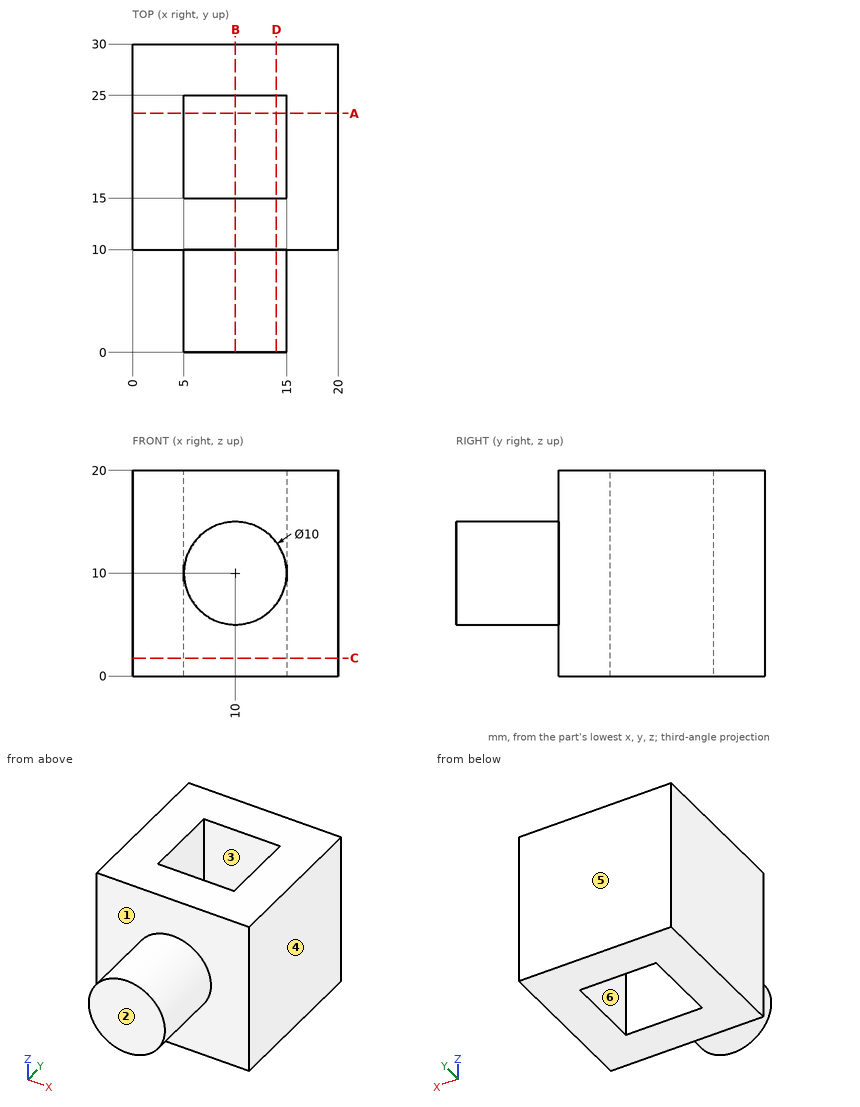
The drawing under review shows one solid part. Ordinate dimensions are in mm from its lowest x, y, z. A direction names the side the tool comes from. Round coordinates to 2 decimals unless told otherwise and drop trailing zeros. Write each loop counter-clockwise with the first axis right and the second up, starting at its lowest first coordinate (ties: lowest second). Pieces come first, ordered by that corner, then holes. Notation, with made-up numbers: (79, 58) - (119, 58) arc R23 cw to (119, 74) - close; hole circle Ø11 at (14.25, 10.25). An arc over 180 degrees is marked (long way). Use one line per item in the form item = value.
Q1. For line 1 (X direction, y = 20.75, z = 11); line 2 (Y direction, x = 9, z = 14); line 3 (Y direction, x = 7, z = 5.5), list the stretches that pass through material, from the lowest coordinate up. Write a range as [from, to].
Answer key:
line_1 = [0, 5], [15, 20]
line_2 = [0, 15], [25, 30]
line_3 = [10, 15], [25, 30]
Q2. Consider section C-C (z = 1.75). State the section outline as (x, y) points, and give its area (3 significant figures).
Answer key:
outline = (0, 10) - (20, 10) - (20, 30) - (0, 30) - close; hole (5, 15) - (15, 15) - (15, 25) - (5, 25) - close
area = 300 mm2
Q3. Consider section D-D (x = 14). State the section outline as (y, z) points.
Answer key:
outline = (0, 7) - (10, 7) - (10, 0) - (15, 0) - (15, 20) - (10, 20) - (10, 13) - (0, 13) - close; (25, 0) - (30, 0) - (30, 20) - (25, 20) - close
Q4. Insertion check: pin 1 Ø3 at (x, y) = (9, 17) entering from +Z. The pin has a flat end and moves straight along its axis. Give the tip position at first contact, or say it passes through.
Answer key:
pin_1 = through
Q5. Draft analysis for pull direction Y (two halves, no side actions). For the marked faces 4, 5 and 6, state which applies: +Y half, -Y half, draft (parallel to the pull), parting line (faces both ways), or undercut.
Answer key:
face_4 = draft
face_5 = +Y half
face_6 = undercut
Q6. Consider section A-A (y = 23.25). State the section outline as (x, z) points.
Answer key:
outline = (0, 0) - (5, 0) - (5, 20) - (0, 20) - close; (15, 0) - (20, 0) - (20, 20) - (15, 20) - close
Q7. Consider section B-B (x = 10). State the section outline as (y, z) points, and give its area (3 significant figures).
Answer key:
outline = (0, 5) - (10, 5) - (10, 0) - (15, 0) - (15, 20) - (10, 20) - (10, 15) - (0, 15) - close; (25, 0) - (30, 0) - (30, 20) - (25, 20) - close
area = 300 mm2
Q8. Tool access review of the marked faces 1, 2 and 3: name each direction out of +Z, -Z, +X, -X, +Y, -Y from which nothing blocks a thin tool from reaching the whole face with its end or side.
Answer key:
face_1 = -Y
face_2 = +Z, -Z, +X, -X, -Y
face_3 = +Z, -Z
